Check sheet for the modelled part. Datum: model origin and axes. Units: mm. A direction names the side the tool comes from. Give positions to 0.01 mm unless a question says otherwise; leave off trailing zeros. Write each loop counter-clockwise with the first axis right and the second up, starting at its lowest first coordinate (ties: lowest second). Pieces come first, ordered by that corner, then holes. Notation, with made-up numbers: M 34.25,1 L 59.25,1 A25 cw 59.25,32 Z; hole C 17.5,39.5 d5. An arc over 180 degrees is marked long. Use CSV: the item, a comma, the result in double quotes. Start each with the question number.
1. Depth check by flat-ended pin: P1, Ø0.8, axis at y = -5.5, z = -4.5, coming from the +X side; P2, Ø5, axis at x = -1, z = 72, coming from the -Y side; P3, Ø2.5, axis at x = 1.5, z = -61.5, coming from the +Y side; P4, Ø1, axis at y = -4, z = -63, coming from the +X side. Enter the tip coordinate at first touch or a pass-through.
2. Mould release check, pull along Z, two halves, no side actions. Record for faces 4 (the face through (0, -6, 90)), 5 (the face through (0.099, -8.352, -57.752)), 6 (the face through (-3.905, -2.268, -0.867)), 7 (the face through (0, -12, -30)): +Z half, -Z half, draft (parallel to the pull), parting line (faces both ways), or undercut.
3. Access from +Z, -Z, +X, -X, +Y, -Y to the whole of each face (thin tool, end or side, straight path). Record for faces 1 (the face through (0.099, -8.352, 62.248)), 2 (the face through (1.201, -2.268, 63.815)), 3 (the face through (0, -12, -75)).
4. Scan lines: line 1 (Z direction, x = 0, y = -8.5); line 2 (Z direction, x = -2.75, y = -3.75); line 3 (X direction, y = -1.8, z = 60). Record each from-to range of solid material in increasing order.
5. Cross-section at A-A, the plane x = 0. Enter the section's corners in (y, z).
from build123d import *

# Parameters (mm, degrees)
EXTRUDE_1_DEPTH           = 90
HOLE_WIZARD_1_D           = 4.5
HOLE_WIZARD_1_CBORE_D     = 8
HOLE_WIZARD_1_CBORE_DEPTH = 4.6
PATTERN_LINEAR_2_COUNT    = 3
PATTERN_LINEAR_2_PITCH    = 60


with BuildPart() as part:
    # 草图1 → 凸台-拉伸1 (new, symmetric)
    with BuildSketch(Plane.XY):
        with BuildLine():
            Line((-7.5, -9.662591907), (-7.5, -11.5))
            Line((-7.5, -11.5), (-6.5, -12.5))
            Line((-6.5, -12.5), (-2.25, -12.5))
            Line((-2.25, -12.5), (-2.25, -12))
            Line((-2.25, -12), (2.25, -12))
            Line((2.25, -12), (2.25, -12.5))
            Line((2.25, -12.5), (6.5, -12.5))
            Line((6.5, -12.5), (7.5, -11.5))
            Line((7.5, -11.5), (7.5, -9.662591907))
            ThreePointArc((7.5, -9.662591907), (7.475491336, -9.507969821), (7.404368042, -9.368506058))
            Line((7.404368042, -9.368506058), (5.691263916, -7.012987884))
            ThreePointArc((5.691263916, -7.012987884), (5.549017328, -6.734060358), (5.5, -6.424816186))
            Line((5.5, -6.424816186), (5.5, -4.75))
            ThreePointArc((5.5, -4.75), (5.552786405, -4.526393202), (5.7, -4.35))
            Line((5.7, -4.35), (5.9371477, -4.172139225))
            ThreePointArc((5.9371477, -4.172139225), (6.03522297, -4.074688525), (6.102860772, -3.954104425))
            ThreePointArc((6.102860772, -3.954104425), (6.504739846, -3.377744581), (7.12499999, -3.047631248))
            ThreePointArc((7.12499999, -3.047631248), (7.395284704, -2.869694549), (7.5, -2.563508327))
            Line((7.5, -2.563508327), (7.5, -1.936491673))
            ThreePointArc((7.5, -1.936491673), (7.395284705, -1.630305452), (7.124999991, -1.452368753))
            ThreePointArc((7.124999991, -1.452368753), (6.439339825, -1.060660169), (6.047631245, -0.375))
            ThreePointArc((6.047631245, -0.375), (5.869694545, -0.104715292), (5.563508327, 0))
            Line((5.563508327, 0), (-5.563508327, 0))
            ThreePointArc((-5.563508327, 0), (-5.869694545, -0.104715292), (-6.047631245, -0.375))
            ThreePointArc((-6.047631245, -0.375), (-6.439339824, -1.060660168), (-7.12499999, -1.452368752))
            ThreePointArc((-7.12499999, -1.452368752), (-7.395284704, -1.630305451), (-7.5, -1.936491673))
            Line((-7.5, -1.936491673), (-7.5, -2.563508327))
            ThreePointArc((-7.5, -2.563508327), (-7.395284705, -2.869694548), (-7.124999991, -3.047631247))
            ThreePointArc((-7.124999991, -3.047631247), (-6.504739849, -3.377744578), (-6.102860775, -3.954104419))
            ThreePointArc((-6.102860775, -3.954104419), (-6.035222972, -4.074688523), (-5.9371477, -4.172139225))
            Line((-5.9371477, -4.172139225), (-5.7, -4.35))
            ThreePointArc((-5.7, -4.35), (-5.552786405, -4.526393202), (-5.5, -4.75))
            Line((-5.5, -4.75), (-5.5, -6.424816186))
            ThreePointArc((-5.5, -6.424816186), (-5.549017328, -6.734060358), (-5.691263916, -7.012987884))
            Line((-5.691263916, -7.012987884), (-7.404368042, -9.368506058))
            ThreePointArc((-7.404368042, -9.368506058), (-7.475491336, -9.507969821), (-7.5, -9.662591907))
        make_face()
    extrude(amount=EXTRUDE_1_DEPTH, both=True)

    # 打孔尺寸(%根据)内六角圆柱头螺钉的类型1 (through all)
    with Locations(Plane(origin=(0, 0, -60), x_dir=(0, 0, 1), z_dir=(0, 1, 0))):
        with Locations((0, 0)):
            hole_wizard_1 = CounterBoreHole(HOLE_WIZARD_1_D / 2, HOLE_WIZARD_1_CBORE_D / 2, HOLE_WIZARD_1_CBORE_DEPTH)

    # 阵列(线性)2: 打孔尺寸(%根据)内六角圆柱头螺钉的类型1 ×3
    with Locations(*[(0, 0, i * PATTERN_LINEAR_2_PITCH) for i in range(1, PATTERN_LINEAR_2_COUNT)]):
        add(hole_wizard_1, mode=Mode.SUBTRACT)


solid = part.part
Worked answers:
1,P1,"stops at x = 5.5"
1,P2,"stops at y = -12.5"
1,P3,"stops at y = -4.6"
1,P4,"stops at x = 6.38"
2,face 4,"+Z half"
2,face 5,"undercut"
2,face 6,"undercut"
2,face 7,"draft"
3,face 1,"+Y, -Y"
3,face 2,"+Y"
3,face 3,"+Z, -Z, -Y"
4,line 1,"z = -90 to -62.25, -57.75 to -2.25, 2.25 to 57.75, 62.25 to 90"
4,line 2,"z = -90 to -62.9, -57.1 to -2.9, 2.9 to 57.1, 62.9 to 90"
4,line 3,"x = -7.48 to -4, 4 to 7.48"
5,outline,"M -12,-90 L 0,-90 L 0,-64 L -4.6,-64 L -4.6,-62.25 L -12,-62.25 Z; M -12,-57.75 L -4.6,-57.75 L -4.6,-56 L 0,-56 L 0,-4 L -4.6,-4 L -4.6,-2.25 L -12,-2.25 Z; M -12,2.25 L -4.6,2.25 L -4.6,4 L 0,4 L 0,56 L -4.6,56 L -4.6,57.75 L -12,57.75 Z; M -12,62.25 L -4.6,62.25 L -4.6,64 L 0,64 L 0,90 L -12,90 Z"
